Build history of the part. All positions in model axes, mm. Face numbers are marked on the shaded views. A direction names the side the tool comes from. Give positions to 0.01 mm unless a question says otherwise; leave off trailing zeros. Order: outer loops, then holes, each group sorted by start corner. A loop starts at its lowest first (then second) coordinate and runs counter-clockwise, first axis right, second up. Notation, with made-up numbers: (29, -12.5) - (74, -12.5) arc R31 ccw to (74, 20.5) - close; hole circle Ø5 at (71.5, -28). An arc over 180 degrees is marked (long way). Use a Markdown table: item, result.
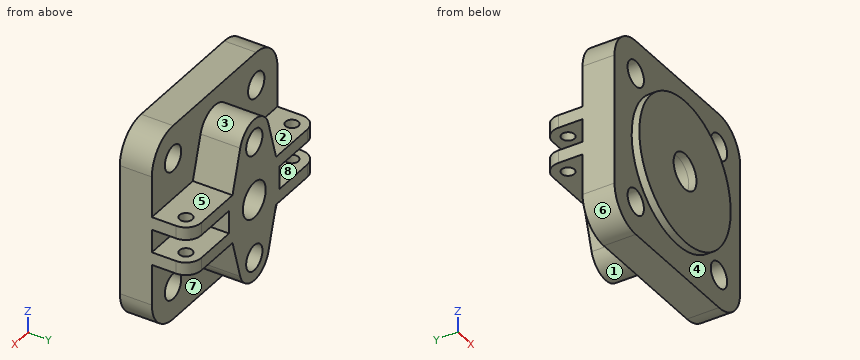
from build123d import *

# Parameters (mm, degrees)
BASE_PLATE_SKETCH_R                  = 10
BASE_PLATE_154X154_DEPTH             = 25
CENTRE_BORE_SKETCH_R                 = 14
CENTRE_BORE_28_DEPTH                 = 25
LOWER_RING_BOSS_SKETCH_R             = 56
LOWER_RING_BOSS_SKETCH_R_2           = 14
LOWER_RING_BOSS_112_DEPTH            = 6
CENTRAL_START                        = 31
CENTRAL_BOSS_SKETCH_R                = 20
CENTRAL_BOSS_SKETCH_R_2              = 14
CENTRAL_BOSS_40_DEPTH                = 31
CROSS_START                          = 31
CROSS_ARMS_SKETCH_R                  = 10
CROSS_ARMS_SKETCH_R_2                = 20
CROSS_ARMS_DEPTH                     = 31
ARM_SLOT_SKETCH_R                    = 10
ARM_SLOT_CUT_DRAFTED_DEPTH           = 22
ARM_SLOT_CUT_DRAFTED_DRAFT           = -2
ARM_SLOT_CUT_DRAFTED_PROFILE_2_DEPTH = 22
ARM_SLOT_CUT_DRAFTED_PROFILE_2_DRAFT = -2
CLEVIS_LUGS_SKETCH_R                 = 5
CLEVIS_LUGS_DEPTH                    = 19
ARM_POCKETS_SKETCH_W                 = 12
ARM_POCKETS_SKETCH_H                 = 18
ARM_POCKETS_AND_HOLES_DEPTH          = 31


with BuildPart() as part:
    # Base Plate Sketch → Base Plate 154x154 (new body)
    with BuildSketch(Plane(origin=(0, 0, 0), x_dir=(1, 0, 0), z_dir=(0, 1, 0))):
        with BuildLine():
            Line((-51, 77), (51, 77))
            ThreePointArc((51, 77), (69.384776311, 69.384776311), (77, 51))
            Line((77, 51), (77, -51))
            ThreePointArc((77, -51), (69.384776311, -69.384776311), (51, -77))
            Line((51, -77), (-51, -77))
            ThreePointArc((-51, -77), (-69.384776311, -69.384776311), (-77, -51))
            Line((-77, -51), (-77, 51))
            ThreePointArc((-77, 51), (-69.384776311, 69.384776311), (-51, 77))
        make_face()
        with Locations(Location((-51, 51, 0), (0, 0, 270))):
            Circle(BASE_PLATE_SKETCH_R, mode=Mode.SUBTRACT)
        with Locations(Location((51, 51, 0), (0, 0, 270))):
            Circle(BASE_PLATE_SKETCH_R, mode=Mode.SUBTRACT)
        with Locations(Location((51, -51, 0), (0, 0, 270))):
            Circle(BASE_PLATE_SKETCH_R, mode=Mode.SUBTRACT)
        with Locations(Location((-51, -51, 0), (0, 0, 270))):
            Circle(BASE_PLATE_SKETCH_R, mode=Mode.SUBTRACT)
    extrude(amount=BASE_PLATE_154X154_DEPTH)

    # Centre Bore Sketch → Centre Bore Ø28 (cut)
    with BuildSketch(Plane(origin=(0, 25, 0), x_dir=(1, 0, 0), z_dir=(0, 1, 0))):
        with Locations(Location((0, 0, 0), (0, 0, 270))):
            Circle(CENTRE_BORE_SKETCH_R)
    extrude(amount=-CENTRE_BORE_28_DEPTH, mode=Mode.SUBTRACT)

    # Lower Ring Boss Sketch → Lower Ring Boss Ø112 (add)
    with BuildSketch(Plane.XZ):
        with Locations(Location((0, 0, 0), (0, 0, 270))):
            Circle(LOWER_RING_BOSS_SKETCH_R)
        with Locations(Location((0, 0, 0), (0, 0, 90))):
            Circle(LOWER_RING_BOSS_SKETCH_R_2, mode=Mode.SUBTRACT)
    extrude(amount=LOWER_RING_BOSS_112_DEPTH)

    # Central Boss Sketch → Central Boss Ø40 (add)
    with BuildSketch(Plane(origin=(0, 25, 0), x_dir=(1, 0, 0), z_dir=(0, 1, 0)).offset(CENTRAL_START)):
        with Locations(Location((0, 0, 0), (0, 0, 270))):
            Circle(CENTRAL_BOSS_SKETCH_R)
        with Locations(Location((0, 0, 0), (0, 0, 270))):
            Circle(CENTRAL_BOSS_SKETCH_R_2, mode=Mode.SUBTRACT)
    extrude(amount=-CENTRAL_BOSS_40_DEPTH)

    # Cross Arms Sketch → Cross Arms (add)
    with BuildSketch(Plane(origin=(0, 25, 0), x_dir=(1, 0, 0), z_dir=(0, 1, 0)).offset(CROSS_START)):
        with BuildLine():
            Line((-29.736293724, 8.760869565), (-17.266235066, 51.086956522))
            ThreePointArc((-17.266235066, 51.086956522), (0, 64), (17.266235066, 51.086956522))
            Line((17.266235066, 51.086956522), (29.736293724, 8.760869565))
            ThreePointArc((29.736293724, 8.760869565), (31, 0), (29.736293724, -8.760869565))
            Line((29.736293724, -8.760869565), (17.266235066, -51.086956522))
            ThreePointArc((17.266235066, -51.086956522), (0, -64), (-17.266235066, -51.086956522))
            Line((-17.266235066, -51.086956522), (-29.736293724, -8.760869565))
            ThreePointArc((-29.736293724, -8.760869565), (-31, 0), (-29.736293724, 8.760869565))
        make_face()
        with Locations(Location((0, 46, 0), (0, 0, 270))):
            Circle(CROSS_ARMS_SKETCH_R, mode=Mode.SUBTRACT)
        with Locations(Location((0, -46, 0), (0, 0, 270))):
            Circle(CROSS_ARMS_SKETCH_R, mode=Mode.SUBTRACT)
        Circle(CROSS_ARMS_SKETCH_R_2, mode=Mode.SUBTRACT)
    extrude(amount=-CROSS_ARMS_DEPTH)


with BuildPart() as arm_slot_cut_drafted_tool:
    # Arm Slot Sketch → Arm Slot Cut Drafted (with draft: the straight prism first)
    with BuildSketch(Plane(origin=(0, 25, 0), x_dir=(1, 0, 0), z_dir=(0, 1, 0))):
        with Locations(Location((0, 46, 0), (0, 0, 270))):
            Circle(ARM_SLOT_SKETCH_R)
    extrude(amount=-ARM_SLOT_CUT_DRAFTED_DEPTH)
    # Arm Slot Cut Drafted: the draft: its side faces are tilted about the plane it starts from
    arm_slot_cut_drafted_sides = [arm_slot_cut_drafted_tool.faces().sort_by_distance(p)[0] for p in [
        (0, 14, -56),
    ]]
    draft(arm_slot_cut_drafted_sides, Plane(origin=(0, 25, 0), x_dir=(1, 0, 0), z_dir=(0, 1, 0)), ARM_SLOT_CUT_DRAFTED_DRAFT)


with BuildPart() as part_1:
    add(part.part)

    # Arm Slot Cut Drafted: cut by arm_slot_cut_drafted_tool
    add(arm_slot_cut_drafted_tool.part, mode=Mode.SUBTRACT)


with BuildPart() as arm_slot_cut_drafted_profile_2_tool:
    # Arm Slot Sketch → Arm Slot Cut Drafted profile 2 (with draft: the straight prism first)
    with BuildSketch(Plane(origin=(0, 25, 0), x_dir=(1, 0, 0), z_dir=(0, 1, 0))):
        with Locations(Location((0, -46, 0), (0, 0, 270))):
            Circle(ARM_SLOT_SKETCH_R)
    extrude(amount=-ARM_SLOT_CUT_DRAFTED_PROFILE_2_DEPTH)
    # Arm Slot Cut Drafted profile 2: the draft: its side faces are tilted about the plane it starts from
    arm_slot_cut_drafted_profile_2_sides = [arm_slot_cut_drafted_profile_2_tool.faces().sort_by_distance(p)[0] for p in [
        (0, 14, 36),
    ]]
    draft(arm_slot_cut_drafted_profile_2_sides, Plane(origin=(0, 25, 0), x_dir=(1, 0, 0), z_dir=(0, 1, 0)), ARM_SLOT_CUT_DRAFTED_PROFILE_2_DRAFT)


with BuildPart() as part_2:
    add(part_1.part)

    # Arm Slot Cut Drafted profile 2: cut by arm_slot_cut_drafted_profile_2_tool
    add(arm_slot_cut_drafted_profile_2_tool.part, mode=Mode.SUBTRACT)

    # Clevis Lugs Sketch → Clevis Lugs (add, symmetric)
    # profile 1 of 2: a face of its own
    with BuildSketch(Plane.XY):
        with BuildLine():
            Line((-19.336072892, 56), (-65, 56))
            ThreePointArc((-65, 56), (-73.485281374, 52.485281374), (-77, 44))
            Line((-77, 44), (-77, 25))
            Line((-77, 25), (-19.336072892, 25))
            Line((-19.336072892, 25), (-19.336072892, 56))
        make_face()
        with Locations((-65, 44)):
            Circle(CLEVIS_LUGS_SKETCH_R, mode=Mode.SUBTRACT)
    # profile 2 of 2: a face of its own
    with BuildSketch(Plane.XY):
        with BuildLine():
            Line((77, 25), (77, 44))
            ThreePointArc((77, 44), (73.485281374, 52.485281374), (65, 56))
            Line((65, 56), (20.121294127, 56))
            Line((20.121294127, 56), (20.121294127, 25))
            Line((20.121294127, 25), (77, 25))
        make_face()
        with Locations((65, 44)):
            Circle(CLEVIS_LUGS_SKETCH_R, mode=Mode.SUBTRACT)
    extrude(amount=CLEVIS_LUGS_DEPTH, both=True)

    # Arm Pockets Sketch → Arm Pockets and Holes (cut)
    with BuildSketch(Plane(origin=(0, 56, 0), x_dir=(1, 0, 0), z_dir=(0, 1, 0))):
        Polygon((-31, 9), (-65, 9), (-65, -9), (-31, -9), (-31, 0), align=None)
        with Locations((-71, 0)):
            Rectangle(ARM_POCKETS_SKETCH_W, ARM_POCKETS_SKETCH_H)
        Polygon((31, 9), (31, 0), (31, -9), (65, -9), (65, 9), align=None)
        with Locations((71, 0)):
            Rectangle(ARM_POCKETS_SKETCH_W, ARM_POCKETS_SKETCH_H)
    extrude(amount=-ARM_POCKETS_AND_HOLES_DEPTH, mode=Mode.SUBTRACT)


solid = part_2.part
1) Tool access for the marked faces 1, 2, 3, 4 and 5: list every direction of +Z, -Z, +X, -X, +Y, -Y with a clear straight run to the whole face (end or side of a thin tool).
Computed:
| item | result |
|---|---|
| face 1 | -Z, +Y |
| face 2 | +Z, -X, +Y |
| face 3 | +Z, +Y |
| face 4 | -Y |
| face 5 | +Z, +X, +Y |
2) Slice it at A-A (z = 0). Write the cut outline in (x, y), and give its area (3 significant figures).
Computed:
| item | result |
|---|---|
| outline | (-77, 0) - (-56, 0) - (-56, -6) - (-14, -6) - (-14, 56) - (-31, 56) - (-31, 25) - (-77, 25) - close; (14, -6) - (56, -6) - (56, 0) - (77, 0) - (77, 25) - (31, 25) - (31, 56) - (14, 56) - close |
| area | 4,710 mm² |
3) Pin check, flat tips, straight feed: P1, Ø15.5, axis at x = 44.5, y = 41.5, coming from the -Z side; P2, Ø9.5, axis at x = 59.5, y = 44.5, coming from the +Z side; P3, Ø5.5, axis at x = -61.5, z = -4, coming from the +Y side. Stop position of each tip, or through.
Computed:
| item | result |
|---|---|
| P1 | stops at z = -19 |
| P2 | stops at z = 19 |
| P3 | stops at y = 25 |
4) Two-plate mould, pull along Z, no slides. Class the marked faces 6, 7 and 8: +Z half, -Z half, draft (parallel to the pull), parting line (faces both ways), or undercut.
Computed:
| item | result |
|---|---|
| face 6 | -Z half |
| face 7 | draft |
| face 8 | undercut |
5) Slice it at D-D (z = -46). Write the cut outline in (x, y).
Computed:
| item | result |
|---|---|
| outline | (-77, 0) - (-59.66, 0) - (-59.66, 25) - (-77, 25) - close; (-42.34, 0) - (-31.94, 0) - (-31.94, -6) - (31.94, -6) - (31.94, 0) - (42.34, 0) - (42.34, 25) - (18.76, 25) - (18.76, 56) - (10, 56) - (10, 25) - (9.23, 3) - (-9.23, 3) - (-10, 25) - (-10, 56) - (-18.76, 56) - (-18.76, 25) - (-42.34, 25) - close; (59.66, 0) - (77, 0) - (77, 25) - (59.66, 25) - close |
6) Slice it at C-C (y = 31). Write the cut outline in (x, z).
Computed:
| item | result |
|---|---|
| outline | (-77, -19) - (-26.72, -19) - (-17.27, -51.09) arc R18 ccw to (17.27, -51.09) - (26.72, -19) - (77, -19) - (77, -9) - (31, -9) - (31, 9) - (77, 9) - (77, 19) - (26.72, 19) - (17.27, 51.09) arc R18 ccw to (-17.27, 51.09) - (-26.72, 19) - (-77, 19) - (-77, 9) - (-31, 9) - (-31, -9) - (-77, -9) - close; hole circle Ø28 at (0, 0); hole circle Ø20 at (0, -46); hole circle Ø20 at (0, 46) |
7) Wall check: line 1 (Z direction, x = -40, y = 52.5); line 2 (X direction, y = 44, z = -16.25); line 3 (X direction, y = 15, z = -51). Give the ranges that are in metal, low to high. Write a range as from..to.
Computed:
| item | result |
|---|---|
| line 1 | z = -19..-9, 9..19 |
| line 2 | x = -77..-70, -60..60, 70..77 |
| line 3 | x = -77..-61, -41..-8.25, 8.25..41, 61..77 |
8) Slice it at B-B (x = 0). Write the cut outline in (y, z), and give its area (3 significant figures).
Computed:
| item | result |
|---|---|
| outline | (-6, -56) - (0, -56) - (0, -77) - (25, -77) - (25, -64) - (56, -64) - (56, -56) - (25, -56) - (3, -55.23) - (3, -36.77) - (25, -36) - (56, -36) - (56, -14) - (-6, -14) - close; (-6, 14) - (56, 14) - (56, 36) - (25, 36) - (3, 36.77) - (3, 55.23) - (25, 56) - (56, 56) - (56, 64) - (25, 64) - (25, 77) - (0, 77) - (0, 56) - (-6, 56) - close |
| area | 4,670 mm² |
